The listing builds one solid part. Answer for the finished solid, in the listing's coordinates (mm). Face numbers are marked on the shaded views. Coordinates: 2 decimals unless noted, no trailing zeros. Order: outer loops, then holes, each group sorted by start corner. A loop starts at its lowest first (then second) coordinate and runs counter-clockwise, first axis right, second up. Notation, with made-up numbers: (33.25, 32) -> (86.25, 32) arc R22 cw to (86.25, 45) -> close; hole circle Ø3 at (13, 68). An arc over 180 degrees is marked (long way). Return JSON: item names as keys, results as strings.
from build123d import *

# Parameters (mm, degrees)
EXTRUDE_1_DEPTH        = 6
EXTRUDE_1_2_DEPTH      = 6
EXTRUDE_1_3_DEPTH      = 6
SKETCH_2_R             = 29.5
EXTRUDE_2_DEPTH        = 40
CHAMFER_1_SIZE         = 1
HOLE_WIZARD_M6_1_D     = 5
HOLE_WIZARD_M6_1_DEPTH = 15
HOLE_WIZARD_M6_1_TIP   = 1.502151548
SKETCH_5_R             = 10.5
CUT_EXTRUDE_1_DEPTH    = 1


with BuildPart() as part:
    # Sketch 1 → Extrude 1 (new body)
    with BuildSketch(Plane(origin=(0, 0, 0), x_dir=(1, 0, 0), z_dir=(0, 1, 0))):
        with BuildLine():
            Line((1.03e-07, 29.5), (-35.507041555, 29.5))
            ThreePointArc((-35.507041555, 29.5), (-43.301270189, 25), (-43.301270189, 16))
            Line((-43.301270189, 16), (-25.547749424, -14.749999978))
            ThreePointArc((-25.547749424, -14.749999978), (-25.54774938, 14.750000056), (1.03e-07, 29.5))
        make_face()
    extrude(amount=EXTRUDE_1_DEPTH)



with BuildPart() as body_2:
    # Sketch 1 → Extrude 1 2 (new body)
    with BuildSketch(Plane(origin=(0, 0, 0), x_dir=(1, 0, 0), z_dir=(0, 1, 0))):
        with BuildLine():
            ThreePointArc((25.547749421, -14.749999984), (-3e-09, -29.5), (-25.547749424, -14.749999978))
            Line((-25.547749424, -14.749999978), (-7.794228634, -45.5))
            ThreePointArc((-7.794228634, -45.5), (0, -50), (7.794228634, -45.5))
            Line((7.794228634, -45.5), (25.547749421, -14.749999984))
        make_face()
    extrude(amount=EXTRUDE_1_2_DEPTH)


with BuildPart() as body_3:
    # Sketch 1 → Extrude 1 3 (new body)
    with BuildSketch(Plane(origin=(0, 0, 0), x_dir=(1, 0, 0), z_dir=(0, 1, 0))):
        with BuildLine():
            Line((35.507041555, 29.5), (1.03e-07, 29.5))
            ThreePointArc((1.03e-07, 29.5), (20.859650082, 20.859650009), (29.5, 0))
            ThreePointArc((29.5, 0), (28.494811878, -7.635161822), (25.547749421, -14.749999984))
            Line((25.547749421, -14.749999984), (43.301270189, 16))
            ThreePointArc((43.301270189, 16), (43.301270189, 25), (35.507041555, 29.5))
        make_face()
    extrude(amount=EXTRUDE_1_3_DEPTH)


with BuildPart() as part_1:
    add(part.part)

    add(body_2.part)  # Extrude 2 merges body 2

    add(body_3.part)  # Extrude 2 merges body 3
    # Sketch 2 → Extrude 2 (add)
    with BuildSketch(Plane(origin=(0, 0, 0), x_dir=(1, 0, 0), z_dir=(0, 1, 0))):
        with Locations(Location((0, 0, 0), (0, 0, 90))):
            Circle(SKETCH_2_R)
        with BuildLine():
            Line((6, 19.602295784), (6, 22.902295784))
            Line((6, 22.902295784), (-6, 22.902295784))
            Line((-6, 22.902295784), (-6, 19.602295784))
            ThreePointArc((-6, 19.602295784), (0, -20.5), (6, 19.602295784))
        make_face(mode=Mode.SUBTRACT)
    extrude(amount=EXTRUDE_2_DEPTH)

    # Chamfer 1
    chamfer_1_edges = [part_1.edges().sort_by_distance(p)[0] for p in [
        (0, 0, 20.5),
        (0, 40, 20.5),
    ]]
    chamfer(chamfer_1_edges, length=CHAMFER_1_SIZE)

    # Hole Wizard M6 _1
    with Locations(Plane(origin=(0, 6, 0), x_dir=(1, 0, 0), z_dir=(0, 1, 0))):
        with Locations((-35.507041555, 20.5), (35.507041555, 20.5), (0, -41)):
            Hole(HOLE_WIZARD_M6_1_D / 2, depth=HOLE_WIZARD_M6_1_DEPTH)
            with Locations((0, 0, -(HOLE_WIZARD_M6_1_DEPTH + HOLE_WIZARD_M6_1_TIP / 2))):  # 118° drill point
                Cone(0, HOLE_WIZARD_M6_1_D / 2, HOLE_WIZARD_M6_1_TIP, mode=Mode.SUBTRACT)

    # Sketch 5 → Cut-Extrude 1 (cut)
    with BuildSketch(Plane(origin=(0, 6, 0), x_dir=(1, 0, 0), z_dir=(0, 1, 0))):
        with Locations((-35.507041555, 20.5)):
            Circle(SKETCH_5_R)
        with Locations((35.507041555, 20.5)):
            Circle(SKETCH_5_R)
        with Locations((0, -41)):
            Circle(SKETCH_5_R)
    extrude(amount=-CUT_EXTRUDE_1_DEPTH, mode=Mode.SUBTRACT)


solid = part_1.part
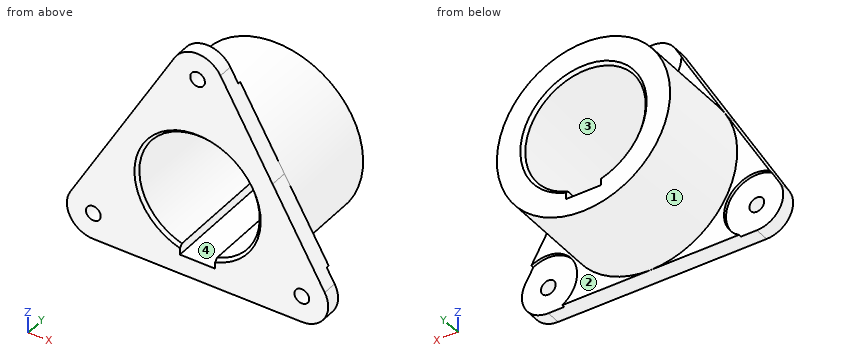
1. Each of these flat-tipped pins is pushed along its axis until it touches: pin 1 Ø2 at (x, y) = (-24.5, 19) entering from -Z; pin 2 Ø3.5 at (x, y) = (1, 19.5) entering from +Z; pin 3 Ø3.5 at (y, z) = (23.5, -21.5) entering from -X. Where does it stop, or does it pass through?
Answer block:
{"pin 1": "stops at z = -17.83", "pin 2": "stops at z = 29.5", "pin 3": "stops at x = -21.91"}
2. The part is cut by section C-C on z = 24.5. Give the vertices of the cut face in (x, y), and give its area (3 significant figures).
Answer block:
{"outline": "(-19.92, 0) -> (19.92, 0) -> (19.92, 6) -> (16.43, 6) -> (16.43, 40) -> (-16.43, 40) -> (-16.43, 6) -> (-19.92, 6) -> close", "area": "1,360 mm2"}
3. The part is cut by section B-B on y = 29. Give the vertices of the cut face in (x, z).
Answer block:
{"outline": "circle Ø59 at (0, 0); hole (-6, -22.9) -> (6, -22.9) -> (6, -19.6) arc R20.5 ccw (long way) to (-6, -19.6) -> close"}
4. Consider line 1 (X direction, y = 1.6, z = -20.5); line 2 (Y direction, x = -28.5, z = -8.5); line 3 (X direction, y = 2, z = -20). Determine where each line is inside the solid, lowest interval first. Write a range as from..to.
Answer block:
{"line 1": "x = -44.51..-38.01, -33.01..-6, 6..33.01, 38.01..44.51", "line 2": "y = 0..6", "line 3": "x = -44.49..-37.96, -33.06..-6, 6..33.06, 37.96..44.49"}
5. The part is cut by section D-D on x = -31.5. Give the vertices of the cut face in (y, z), and give its area (3 significant figures).
Answer block:
{"outline": "(0, -29.5) -> (5, -29.5) -> (5, -10.79) -> (6, -10.79) -> (6, 4.44) -> (0, 4.44) -> close", "area": "185 mm2"}
6. The part is cut by section A-A on z = 0. Give the vertices of the cut face in (x, y), and give its area (3 significant figures).
Answer block:
{"outline": "(-34.06, 0) -> (-21.5, 0) -> (-20.5, 1) -> (-20.5, 39) -> (-21.5, 40) -> (-29.5, 40) -> (-29.5, 6) -> (-34.06, 6) -> close; (20.5, 1) -> (21.5, 0) -> (34.06, 0) -> (34.06, 6) -> (29.5, 6) -> (29.5, 40) -> (21.5, 40) -> (20.5, 39) -> close", "area": "773 mm2"}
7. Determine the mould class of the marked faces 1, 2, 3 and 4 for opening direction X: pulls with the +X half, pulls with the -X half, needs draft (parallel to the pull), parting line crosses it, or undercut.
Answer block:
{"face 1": "parting line crosses it", "face 2": "needs draft", "face 3": "undercut", "face 4": "undercut"}
